from build123d import *

# Parameters (mm, degrees)
BASE_PLATE_SKETCH_W                = 140
BASE_PLATE_SKETCH_H                = 80
BASE_PLATE_140X80X16_DEPTH         = 16
LOWER_COLUMN_SKETCH_R              = 22.5
LOWER_COLUMN_45_DEPTH              = 34
UPPER_COLUMN_SKETCH_R              = 28
UPPER_COLUMN_56_DEPTH              = 40
SIDE_ARM_DEPTH                     = 10
ELBOW_SWEEP_45_PROFILE_R           = 22.5
HEX_NUT_OUTLET_DEPTH               = 15
ARM_BOSS_SKETCH_R                  = 12
ARM_BOSS_24_DEPTH                  = 16
OUTLET_BORE_SKETCH_R               = 17.5
OUTLET_BORE_35_DEPTH               = 56.392557
ELBOW_PROFILE_CUT_PROFILE_R        = 15
FLOW_PASSAGE_12_PROFILE_R          = 6
COLUMN_GROOVE_SKETCH_W             = 25
COLUMN_GROOVE_SKETCH_H             = 30
ARM_BOSS_HOLE_SKETCH_R             = 7
ARM_BOSS_HOLE_14_DEPTH             = 30
BASE_PLATE_CORNER_FILLETS_R15_R    = 15
MOUNTING_HOLES_CBORE_9_D           = 9
MOUNTING_HOLES_CBORE_9_DEPTH       = 19.773719933
MOUNTING_HOLES_CBORE_9_CBORE_D     = 15
MOUNTING_HOLES_CBORE_9_CBORE_DEPTH = 5


with BuildPart() as part:
    # Base Plate Sketch → Base Plate 140x80x16 (new body)
    with BuildSketch(Plane(origin=(0, 0, 0), x_dir=(1, 0, 0), z_dir=(0, 1, 0))):
        Rectangle(BASE_PLATE_SKETCH_W, BASE_PLATE_SKETCH_H)
    extrude(amount=BASE_PLATE_140X80X16_DEPTH)

    # Lower Column Sketch → Lower Column _45 (add)
    with BuildSketch(Plane(origin=(0, 16, 0), x_dir=(1, 0, 0), z_dir=(0, 1, 0))):
        with Locations(Location((0, 0, 0), (0, 0, 270))):
            Circle(LOWER_COLUMN_SKETCH_R)
    extrude(amount=LOWER_COLUMN_45_DEPTH)

    # Upper Column Sketch → Upper Column _56 (add)
    with BuildSketch(Plane(origin=(0, 50, 0), x_dir=(1, 0, 0), z_dir=(0, 1, 0))):
        with Locations(Location((0, 0, 0), (0, 0, 270))):
            Circle(UPPER_COLUMN_SKETCH_R)
    extrude(amount=UPPER_COLUMN_56_DEPTH)

    # Side Arm Sketch → Side Arm (add, symmetric)
    with BuildSketch(Plane(origin=(0, 70, 0), x_dir=(1, 0, 0), z_dir=(0, 1, 0))):
        with BuildLine():
            Line((-84.37804878, 14.810296553), (-4.43902439, 27.6458869))
            ThreePointArc((-4.43902439, 27.6458869), (-28, 0), (-4.43902439, -27.6458869))
            Line((-4.43902439, -27.6458869), (-84.37804878, -14.810296553))
            ThreePointArc((-84.37804878, -14.810296553), (-97, 0), (-84.37804878, 14.810296553))
        make_face()
    extrude(amount=SIDE_ARM_DEPTH, both=True)

    # Elbow Sweep _45: sweep along a path in Elbow Path Sketch
    with BuildLine(Plane.XY) as elbow_sweep_45_path:
        Line((0, 0), (0, 104.392557166))
        ThreePointArc((0, 104.392557166), (3.238590518, 118.420433863), (12.29883279, 129.608901281))
        Line((12.29883279, 129.608901281), (56.73677426, 164.327626223))
    # Elbow Sweep _45 profile (on start of the path) → Elbow Sweep _45 (sweep)
    with BuildSketch(Plane.ZX):
        Circle(ELBOW_SWEEP_45_PROFILE_R)
    sweep(path=elbow_sweep_45_path.line)

    # Hex Nut Sketch → Hex Nut Outlet (add)
    with BuildSketch(Plane(origin=(111.014464068, 86.734005111, 0), x_dir=(0, 0, -1), z_dir=(0.7880107536067209, 0.6156614753256597, 0))):
        Polygon((-38.682468036, 94.561290433), (-19.341234018, 61.061290433), (19.341234018, 61.061290433), (38.682468036, 94.561290433), (19.341234018, 128.061290433), (-19.341234018, 128.061290433), align=None)
    extrude(amount=-HEX_NUT_OUTLET_DEPTH)

    # Arm Boss Sketch → Arm Boss _24 (add)
    with BuildSketch(Plane(origin=(0, 80, 0), x_dir=(1, 0, 0), z_dir=(0, 1, 0))):
        with Locations(Location((-82, 0, 0), (0, 0, 270))):
            Circle(ARM_BOSS_SKETCH_R)
    extrude(amount=ARM_BOSS_24_DEPTH)

    # Outlet Bore Sketch → Outlet Bore _35 (cut)
    with BuildSketch(Plane(origin=(114.954517836, 89.812312487, 0), x_dir=(0, 0, -1), z_dir=(0.7880107536067209, 0.6156614753256597, 0))):
        with Locations(Location((0, 94.561290433, 0), (0, 0, 90))):
            Circle(OUTLET_BORE_SKETCH_R)
    extrude(amount=-OUTLET_BORE_35_DEPTH, mode=Mode.SUBTRACT)

    # Elbow Profile Cut: sweep along a path in Elbow Profile Cut Sketch
    with BuildLine(Plane.XY) as elbow_profile_cut_path:
        Line((56.73677426, 164.327626223), (12.29883279, 129.608901281))
        ThreePointArc((12.29883279, 129.608901281), (7.332840345, 124.777140423), (3.523289487, 118.989712997))
    # Elbow Profile Cut profile (on start of the path) → Elbow Profile Cut (sweep, cut)
    with BuildSketch(Plane(origin=(56.73677426, 164.327626223, 0), x_dir=(0.6156614753256594, -0.7880107536067211, 0), z_dir=(-0.7880107536067211, -0.6156614753256594, 0))):
        Circle(ELBOW_PROFILE_CUT_PROFILE_R)
    sweep(path=elbow_profile_cut_path.line, mode=Mode.SUBTRACT)

    # Flow Passage _12: sweep along a path in Sketch5_4
    with BuildLine(Plane.XY) as flow_passage_12_path:
        Line((0, 0), (0, 104.392557166))
        ThreePointArc((0, 104.392557166), (3.238590518, 118.420433863), (12.29883279, 129.608901281))
        Line((12.29883279, 129.608901281), (56.73677426, 164.327626223))
    # Flow Passage _12 profile (on start of the path) → Flow Passage _12 (sweep, cut)
    with BuildSketch(Plane.ZX):
        Circle(FLOW_PASSAGE_12_PROFILE_R)
    sweep(path=flow_passage_12_path.line, mode=Mode.SUBTRACT)

    # Column Groove Sketch → Column Groove (revolve, cut)
    with BuildSketch(Plane.XY):
        with Locations((-12.5, 70)):
            Rectangle(COLUMN_GROOVE_SKETCH_W, COLUMN_GROOVE_SKETCH_H)
    revolve(axis=Axis((0, 55, 0), (0, 1, 0)), mode=Mode.SUBTRACT)

    # Arm Boss Hole Sketch → Arm Boss Hole _14 (cut)
    with BuildSketch(Plane(origin=(0, 96, 0), x_dir=(1, 0, 0), z_dir=(0, 1, 0))):
        with Locations(Location((-82, 0, 0), (0, 0, 270))):
            Circle(ARM_BOSS_HOLE_SKETCH_R)
    extrude(amount=-ARM_BOSS_HOLE_14_DEPTH, mode=Mode.SUBTRACT)

    # Base Plate Corner Fillets R15
    base_plate_corner_fillets_r15_edges = [part.edges().sort_by_distance(p)[0] for p in [
        (70, 8, 40),
        (-70, 8, 40),
        (-70, 8, -40),
        (70, 8, -40),
    ]]
    fillet(base_plate_corner_fillets_r15_edges, radius=BASE_PLATE_CORNER_FILLETS_R15_R)

    # Mounting Holes CBore _9
    with Locations(Plane(origin=(0, 16, 0), x_dir=(1, 0, 0), z_dir=(0, 1, 0))):
        with Locations((55, -25), (55, 25), (-56.445631344, 25), (-55, -25)):
            CounterBoreHole(MOUNTING_HOLES_CBORE_9_D / 2, MOUNTING_HOLES_CBORE_9_CBORE_D / 2, MOUNTING_HOLES_CBORE_9_CBORE_DEPTH, depth=MOUNTING_HOLES_CBORE_9_DEPTH)


solid = part.part
For this review, take the finished solid that the model builds, in its own axes (mm). A direction names the side the tool comes from. Give positions to 0.01 mm unless a question says otherwise; leave off trailing zeros. Order: outer loops, then holes, each group sorted by start corner. A loop starts at its lowest first (then second) coordinate and runs counter-clockwise, first axis right, second up. Notation, with made-up numbers: M 64.25,-36.5 L 69.25,-36.5 A25 cw 69.25,-20.5 Z; hole C 63,-5 d3. An arc over 180 degrees is marked long. Answer in a Markdown table with one row per item. Add a question column.
(1) For faces 1 (the face through (52.581, 5.423, -28.794)), 2 (the face through (-82, 66, 0)), 3 (the face through (57.137, 143.682, 29.147)), 4 (the face through (-19.961, 97.297, 10.382)), 5 (the face through (70, 8, 0)), list the 3-axis set-ups (+Z, -Z, +X, -X, +Y, -Y) from which the entire face can be reached by the end or side of a thin tool; tool diameter is ignored.
(2) Consider section B-B on y = 41. State the section outline as (x, z) points, and give its area (3 significant figures).
(3) Wall thickness on probe 1 along Z at (x, y) = (55, 12.95); probe 2 along Z at (x, y) = (55, 5.75); probe 3 along X at (y, z) = (3, -25): over which ranges is each line inside the solid? List them lowest first. Write a range as [from, to].
(4) For pin 1 (17 mm diameter, centred on x = -11.5, z = -4.5, fed in from +Y); pin 2 (5 mm diameter, centred on y = 122.5, z = -27, fed in from +X); pin 3 (7 mm diameter, centred on x = 55, z = 25, fed in from +Y); pin 4 (12 mm diameter, centred on x = -56.45, z = -25, fed in from +Y), all flat-tipped, find the tip position at first contact; note any pin that passes through.
(5) Consider section A-A on x = -82. State the section outline as (y, z) points, and give its area (3 significant figures).
(6) Mouldability with a two-part tool opening along Z and no side actions: class faces 6 (the face through (-1, 8, 40)), 7 (the face through (26.34, 183.09, -0.27)), 8 (the face through (-57.419, 5.423, 21.206)) as +Z half, -Z half, draft (parallel to the pull), parting line (faces both ways), or undercut.
Evaluation:
| question | item | result |
|---|---|---|
| 1 | face 1 | -Y |
| 1 | face 2 | +Y |
| 1 | face 3 | +Z, +X |
| 1 | face 4 | none |
| 1 | face 5 | +Z, -Z, +X, -Y |
| 2 | outline | C 0,0 d45; hole C 0,0 d12 |
| 2 | area | 1,480 mm^2 |
| 3 | probe 1 | z = [-40, -32.5], [-17.5, 17.5], [32.5, 40] |
| 3 | probe 2 | z = [-40, -29.5], [-20.5, 20.5], [29.5, 40] |
| 3 | probe 3 | x = [-70, -60.95], [-51.95, 50.5], [59.5, 70] |
| 4 | pin 1 | stops at y = 145.8 |
| 4 | pin 2 | passes through |
| 4 | pin 3 | stops at y = 168.53 |
| 4 | pin 4 | stops at y = 80 |
| 5 | outline | M 60,-15.19 L 80,-15.19 L 80,-12 L 96,-12 L 96,-7 L 66,-7 L 66,7 L 96,7 L 96,12 L 80,12 L 80,15.19 L 60,15.19 Z |
| 5 | area | 572 mm^2 |
| 6 | face 6 | +Z half |
| 6 | face 7 | draft |
| 6 | face 8 | undercut |
